Build history of the part. All positions in model axes, mm. A direction names the side the tool comes from. Give positions to 0.01 mm unless a question says otherwise; leave off trailing zeros. Order: outer loops, then holes, each group sorted by start corner. A loop starts at its lowest first (then second) coordinate and runs counter-clockwise, first axis right, second up. Notation, with made-up numbers: (-36, -34.75) - (-20, -34.75) arc R18 ccw to (-20, -25.75) - close; hole circle Ø10 at (-17.75, 77). An arc over 180 degrees is marked (long way). Use a Markdown table: item, result. Add a question column.
(1) Slice it at B-B (y = 23). Write the cut outline in (x, z).
(2) Wall check: line 1 (Y direction, x = 0, z = -0.2); line 2 (Y direction, x = 85, z = 1.6); line 3 (X direction, y = -4.5, z = 1). Give the ranges that are in metal, low to high.
(3) Mould opens along Y. For faces 1 (the face through (-48.03, -10.69, -0.05)), 2 (the face through (71.3, -9.5, 0)), 3 (the face through (8.74, 17.59, 0.05)), 4 (the face through (-39.878, 50.058, 0.049)) say: +Y half, -Y half, draft (parallel to the pull), parting line (faces both ways), or undercut.
(4) Slice it at C-C (z = -1.75). Write the cut outline in (x, y) (3 decimals), then the cut area to 3 significant figures.
(5) Which spindle directions (+Z, -Z, +X, -X, +Y, -Y) get a long thin tool onto all of the face, cutting with end or side? Do faces 5 (the face through (44, -9, 0)), 6 (the face through (20, 19, -3.5)), 7 (the face through (-32.91, -8.82, 0.05)). Say none if no direction does.
(6) Slice it at A-A (x = 0). Write the cut outline in (y, z), then the cut area to 4 significant figures.
(7) Slice it at D-D (x = 85). Write the cut outline in (y, z), then the cut area to 4 significant figures.
from build123d import *

# Parameters (mm, degrees)
OPENER_PROFILE_SKETCH_R   = 8
OPENER_PROFILE_SKETCH_R_2 = 10.5
OPENER_PLATE_7MM_DEPTH    = 3.5
EDGE_FILLETS_R6_R         = 6
EDGE_CHAMFERS_0_5X45_SIZE = 0.5


with BuildPart() as part:
    # Opener Profile Sketch → Opener Plate 7mm (new, symmetric)
    with BuildSketch(Plane.XY):
        with BuildLine():
            Line((20.207259422, 9), (71.771243445, 9))
            ThreePointArc((71.771243445, 9), (101, 0), (71.771243445, -9))
            Line((71.771243445, -9), (15.588457268, -9))
            ThreePointArc((15.588457268, -9), (4.846344572, -17.335309178), (-8.66103197, -15.779306867))
            Line((-8.66103197, -15.779306867), (-57.165847871, -28.776133117))
            ThreePointArc((-57.165847871, -28.776133117), (-38.960731457, 50.774613779), (42.591220317, 47.770157545))
            Line((42.591220317, 47.770157545), (20.207259422, 9))
        make_face()
        with Locations((85, 0)):
            Circle(OPENER_PROFILE_SKETCH_R, mode=Mode.SUBTRACT)
        Circle(OPENER_PROFILE_SKETCH_R_2, mode=Mode.SUBTRACT)
        with BuildLine():
            Line((9, 15.588457268), (25.5, 44.167295593))
            ThreePointArc((25.5, 44.167295593), (-31.046832879, 40.461020355), (-49.262217141, -13.1997713))
            Line((-49.262217141, -13.1997713), (-17.386664873, -4.658742812))
            ThreePointArc((-17.386664873, -4.658742812), (-10.957705722, 14.280360125), (9, 15.588457268))
        make_face(mode=Mode.SUBTRACT)
    extrude(amount=OPENER_PLATE_7MM_DEPTH, both=True)

    # Edge Fillets R6
    edge_fillets_r6_edges = [part.edges().sort_by_distance(p)[0] for p in [
        (71.771243445, -9, 0),
        (15.588457268, -9, 0),
        (-8.66103197, -15.779306867, 0),
        (-57.165847871, -28.776133117, 0),
        (42.591220317, 47.770157545, 0),
        (20.207259422, 9, 0),
        (71.771243445, 9, 0),
        (-17.386664873, -4.658742812, 0),
        (9, 15.588457268, 0),
        (25.5, 44.167295593, 0),
        (-49.262217141, -13.1997713, 0),
    ]]
    fillet(edge_fillets_r6_edges, radius=EDGE_FILLETS_R6_R)

    # Edge Chamfers 0.5x45
    edge_chamfers_0_5x45_edges = [part.edges().sort_by_distance(p)[0] for p in [
        (77, 0, -3.5),
        (77, 0, 3.5),
        (-10.5, 0, -3.5),
        (-10.5, 0, 3.5),
    ]]
    chamfer(edge_chamfers_0_5x45_edges, length=EDGE_CHAMFERS_0_5X45_SIZE)


solid = part.part
Solution:
| question | item | result |
|---|---|---|
| 1 | outline | (-59.72, -3.5) - (-45.52, -3.5) - (-45.52, 3.5) - (-59.72, 3.5) - close; (13.28, -3.5) - (28.29, -3.5) - (28.29, 3.5) - (13.28, 3.5) - close |
| 2 | line 1 | -18 to -10.5, 10.5 to 18, 51 to 64 |
| 2 | line 2 | -16 to -8, 8 to 16 |
| 2 | line 3 | -63.84 to -50.8, -19.8 to -9.49, 9.49 to 78.39, 91.61 to 100.35 |
| 3 | face 1 | undercut |
| 3 | face 2 | -Y half |
| 3 | face 3 | undercut |
| 3 | face 4 | parting line |
| 4 | outline | (-59.368, -23.904) arc R6 ccw to (-52.25, -27.459) - (-10.799, -16.352) arc R6 cw to (-6.934, -16.611) arc R18 ccw to (14.051, -11.25) arc R6 cw to (18.735, -9) - (68.907, -9) arc R6 cw to (73.296, -10.909) arc R16 ccw (long way) to (73.296, 10.909) arc R6 cw to (68.907, 9) - (30.6, 9) arc R6 cw to (25.403, 18) - (40.046, 43.362) arc R6 ccw to (38.455, 51.158) arc R64 ccw to start; hole (-50.582, -6.514) arc R6 ccw to (-43.079, -11.543) - (-22.446, -6.014) arc R6 ccw to (-17.999, -0.164) arc R18 cw to (4.817, 17.343) arc R6 ccw to (11.619, 20.125) - (22.299, 38.623) arc R6 ccw to (19.383, 47.173) arc R51 ccw to start; hole circle Ø21 at (0, 0); hole circle Ø16 at (85, 0) |
| 4 | area | 5,250 mm2 |
| 5 | face 5 | +Z, -Z, -Y |
| 5 | face 6 | -Z, +X, -X, +Y, -Y |
| 5 | face 7 | +Z, -Z |
| 6 | outline | (-18, -3.5) - (-11, -3.5) - (-10.5, -3) - (-10.5, 3) - (-11, 3.5) - (-18, 3.5) - close; (10.5, -3) - (11, -3.5) - (18, -3.5) - (18, 3.5) - (11, 3.5) - (10.5, 3) - close; (51, -3.5) - (64, -3.5) - (64, 3.5) - (51, 3.5) - close |
| 6 | area | 195.5 mm2 |
| 7 | outline | (-16, -3.5) - (-8.5, -3.5) - (-8, -3) - (-8, 3) - (-8.5, 3.5) - (-16, 3.5) - close; (8, -3) - (8.5, -3.5) - (16, -3.5) - (16, 3.5) - (8.5, 3.5) - (8, 3) - close |
| 7 | area | 111.5 mm2 |
